Check sheet for the modelled part. Datum: model origin and axes. Units: mm. A direction names the side the tool comes from. Give positions to 0.01 mm unless a question says otherwise; leave off trailing zeros. Write each loop counter-clockwise with the first axis right and the second up, starting at its lowest first coordinate (ties: lowest second). Pieces come first, ordered by that corner, then holes. Notation, with made-up numbers: (52, -4) -> (87, -4) arc R21 cw to (87, 9) -> close; hole circle Ø6 at (47, -39.75). An arc over 180 degrees is marked (long way). Answer as a JSON object with one key per item and string values.
from build123d import *

# Parameters (mm, degrees)
SKETCH1_R               = 30
SKETCH1_R_2             = 24
BOSS_EXTRUDE1_DEPTH     = 30
CUT_EXTRUDE1_DEPTH      = 52.961524227
CUT_EXTRUDE1_DEPTH_BACK = 52.961524227
SKETCH2_W               = 38
SKETCH2_H               = 18


with BuildPart() as part:
    # Sketch1 → Boss-Extrude1 (new body)
    with BuildSketch(Plane(origin=(0, 0, 0), x_dir=(1, 0, 0), z_dir=(0, 1, 0))):
        with Locations(Location((0, 0, 0), (0, 0, 270))):
            Circle(SKETCH1_R)
        with Locations(Location((0, 0, 0), (0, 0, 270))):
            Circle(SKETCH1_R_2, mode=Mode.SUBTRACT)
    extrude(amount=BOSS_EXTRUDE1_DEPTH)

    # Sketch2 → Cut-Extrude1 (cut, two sides: drawn at the far end of the back side and taken through both)
    with BuildSketch(Plane(origin=(0, 0, 0), x_dir=(0, 0, -1), z_dir=(1, 0, 0)).offset(-CUT_EXTRUDE1_DEPTH_BACK)):
        with Locations((-30, 15)):
            Rectangle(SKETCH2_W, SKETCH2_H)
        with Locations((30, 15)):
            Rectangle(SKETCH2_W, SKETCH2_H)
    extrude(amount=CUT_EXTRUDE1_DEPTH + CUT_EXTRUDE1_DEPTH_BACK, mode=Mode.SUBTRACT)


solid = part.part
1. Go/stop test with flat-tipped pins: P1, Ø5.5, axis at x = 25.5, y = 16, coming from the +Z side; P2, Ø1, axis at x = 6.5, z = -22, coming from the +Y side; P3, Ø5.5, axis at x = -23, y = 15.5, coming from the -Z side; P4, Ø6, axis at x = -4.5, y = 3.5, coming from the -Z side. Record where each tip stops, or that it passes through.
Determined:
{"P1": "z = 11", "P2": "through", "P3": "z = -11", "P4": "z = -29.96"}
2. Sectioned sample at A-A, the plane x = 0. Enter the section's corners in (y, z), plus the area to 3 significant figures.
Determined:
{"outline": "(0, -30) -> (6, -30) -> (6, -24) -> (0, -24) -> close; (0, 24) -> (6, 24) -> (6, 30) -> (0, 30) -> close; (24, -30) -> (30, -30) -> (30, -24) -> (24, -24) -> close; (24, 24) -> (30, 24) -> (30, 30) -> (24, 30) -> close", "area": "144 mm^2"}
3. Sectioned sample at B-B, the plane y = 15.75. Enter the section's corners in (x, z), plus the area to 3 significant figures.
Determined:
{"outline": "(-27.91, -11) -> (-21.33, -11) arc R24 cw to (-21.33, 11) -> (-27.91, 11) arc R30 ccw to start; (21.33, -11) -> (27.91, -11) arc R30 ccw to (27.91, 11) -> (21.33, 11) arc R24 cw to start", "area": "272 mm^2"}
4. Sectioned sample at D-D, the plane z = 0. Enter the section's corners in (x, y).
Determined:
{"outline": "(-30, 0) -> (-24, 0) -> (-24, 30) -> (-30, 30) -> close; (24, 0) -> (30, 0) -> (30, 30) -> (24, 30) -> close"}
5. Access from +Z, -Z, +X, -X, +Y, -Y to the whole of each face (thin tool, end or side, straight path). Record for faces 4 (the face through (-25, 15, -11)), 5 (the face through (20.1, 30, -13.5)), 6 (the face through (-25, 15, 11)).
Determined:
{"face 4": "-Z, +X, -X", "face 5": "+Z, -Z, +X, -X, +Y", "face 6": "+Z, +X, -X"}
6. Scan lines: L1, parallel to Y at x = -15.5, z = 21.5; L2, parallel to X at y = 11.5, z = 0; L3, parallel to Z at x = 27, y = 23.5. Record each from-to range of solid material in increasing order. Write a range as [from, to].
Determined:
{"L1": "[0, 6], [24, 30]", "L2": "[-30, -24], [24, 30]", "L3": "[-11, 11]"}
7. Sectioned sample at C-C, the plane z = -12.5. Enter the section's corners in (x, y), plus the area to 3 significant figures.
Determined:
{"outline": "(-27.27, 0) -> (-20.49, 0) -> (-20.49, 6) -> (-27.27, 6) -> close; (-27.27, 24) -> (-20.49, 24) -> (-20.49, 30) -> (-27.27, 30) -> close; (20.49, 0) -> (27.27, 0) -> (27.27, 6) -> (20.49, 6) -> close; (20.49, 24) -> (27.27, 24) -> (27.27, 30) -> (20.49, 30) -> close", "area": "163 mm^2"}
8. Mould release check, pull along X, two halves, no side actions. Record for faces 1 (the face through (-29.287, 14.79, -6.503)), 2 (the face through (-23.43, 14.79, -5.2)), 3 (the face through (20.1, 0, -13.5)): released by +X, released by -X, zero draft, split by the parting line, or undercut.
Determined:
{"face 1": "split by the parting line", "face 2": "undercut", "face 3": "zero draft"}
